The model under review builds one solid part; all positions refer to its coordinate system, in mm. Face numbers are marked on the shaded views. Round coordinates to 2 decimals unless told otherwise and drop trailing zeros. Loops run counter-clockwise (first coordinate to the right, second up) from the corner with the lowest first, then second, coordinate; pieces in that order, holes last. Notation, with made-up numbers: M 1,76.5 L 40,76.5 A18 cw 40,87.5 Z; hole C 35,19 d8. An arc over 180 degrees is marked long. One line per question, with ' | ' between items.
from build123d import *

# Parameters (mm, degrees)
EXTRUDE1_DEPTH          = 5
CUT_EXTRUDE1_DEPTH      = 9.958236434
CUT_EXTRUDE1_DEPTH_BACK = 9.958236434
FILLET2_R               = 0.25


with BuildPart() as part:
    # Sketch1 → Extrude1 (new body)
    with BuildSketch(Plane.XY):
        with BuildLine():
            Line((-7, 2.5), (4.5, 2.5))
            ThreePointArc((4.5, 2.5), (7, 0), (4.5, -2.5))
            Line((4.5, -2.5), (-7, -2.5))
            Line((-7, -2.5), (-7, 2.5))
        make_face()
    extrude(amount=EXTRUDE1_DEPTH)

    # Sketch2 → Cut-Extrude1 (cut, two sides: drawn at the far end of the back side and taken through both)
    with BuildSketch(Plane(origin=(0, 0, 0), x_dir=(1, 0, 0), z_dir=(0, 1, 0)).offset(-CUT_EXTRUDE1_DEPTH_BACK)):
        Polygon((-7, 0), (7, 0), (7, -0.14), align=None)
    extrude(amount=CUT_EXTRUDE1_DEPTH + CUT_EXTRUDE1_DEPTH_BACK, mode=Mode.SUBTRACT)

    # Fillet2
    fillet2_edges = [part.edges().sort_by_distance(p)[0] for p in [
        (7, 0, 5),
        (-1.25, 2.5, 5),
        (-1.25, -2.5, 0.0575),
        (6.267744857, -1.767789049, 0.132677449),
        (-1.25, 2.5, 0.0575),
        (-1.25, -2.5, 5),
    ]]
    fillet(fillet2_edges, radius=FILLET2_R)


solid = part.part
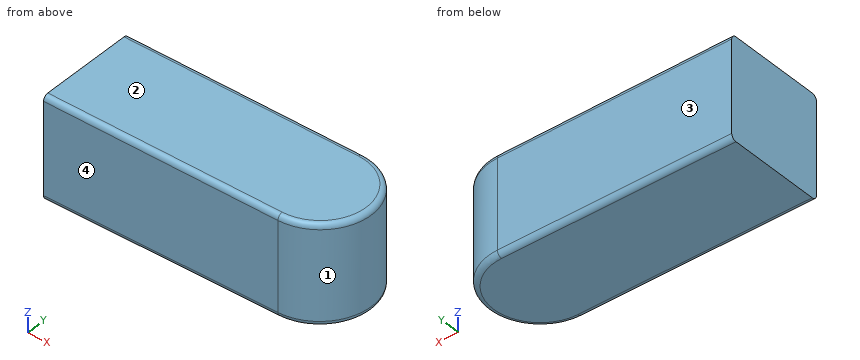
1) Insertion check: P1, Ø1, axis at x = 1, y = -1, coming from the -Z side (3 decimals); P2, Ø1.5, axis at y = -2, z = 2.5, coming from the +X side. Each pin has a flat end and moves straight along its axis. Give the tip position at first contact, or say it passes through.
Output values:
P1: stops at z = 0.075 | P2: stops at x = 6.67
2) Mouldability with a two-part tool opening along Y and no side actions: class the marked faces 1, 2, 3 and 4 as +Y half, -Y half, draft (parallel to the pull), parting line (faces both ways), or undercut.
Output values:
face 1: parting line | face 2: draft | face 3: +Y half | face 4: -Y half
3) Add section A-A on z = 2.55. State the section outline as (x, y) points.
Output values:
outline: M -7,-2.5 L 4.5,-2.5 A2.5 ccw 4.5,2.5 L -7,2.5 Z
4) For line 1 (Z direction, x = 5.5, y = -0.5) (3 decimals); line 2 (X direction, y = 0.2, z = 4.8); line 3 (Y direction, x = 5.75, z = 2.65), list the stretches that pass through material, from the lowest coordinate up.
Output values:
line 1: z = 0.125 to 5 | line 2: x = -7 to 6.99 | line 3: y = -2.17 to 2.17
